from build123d import *

# Parameters (mm, degrees)
BASE_BLOCK_SKETCH_W       = 28
BASE_BLOCK_SKETCH_H       = 48
BASE_BLOCK_DEPTH          = 24
FORK_ARMS_DEPTH           = 10
FORK_ARC_CUT_SKETCH_R33_R = 16.5
FORK_ARC_CUT_DEPTH        = 20
EYE_START                 = -24
EYE_LUG_WITH_BORE_DEPTH   = 10


with BuildPart() as part:
    # Base Block Sketch → Base Block (new, symmetric)
    with BuildSketch(Plane.XY):
        with Locations((14, -24)):
            Rectangle(BASE_BLOCK_SKETCH_W, BASE_BLOCK_SKETCH_H)
    extrude(amount=BASE_BLOCK_DEPTH, both=True)

    # Fork Arms Sketch → Fork Arms (add, symmetric)
    with BuildSketch(Plane(origin=(0, -24, 0), x_dir=(1, 0, 0), z_dir=(0, 1, 0))):
        with BuildLine():
            Line((52, 24), (28, 24))
            Line((28, 24), (28, -24))
            Line((28, -24), (52, -24))
            ThreePointArc((52, -24), (76, 0), (52, 24))
        make_face()
    extrude(amount=FORK_ARMS_DEPTH, both=True)

    # Fork Arc Cut Sketch R33 → Fork Arc Cut (cut)
    with BuildSketch(Plane(origin=(0, -14, 0), x_dir=(1, 0, 0), z_dir=(0, 1, 0))):
        with Locations(Location((52, 0, 0), (0, 0, 270))):
            Circle(FORK_ARC_CUT_SKETCH_R33_R)
    extrude(amount=-FORK_ARC_CUT_DEPTH, mode=Mode.SUBTRACT)

    # Eye Lug Sketch → Eye Lug With Bore (add, symmetric)
    with BuildSketch(Plane.XY.offset(24).offset(EYE_START)):
        with BuildLine():
            Line((0, 0), (-32.031280577, 0))
            ThreePointArc((-32.031280577, 0), (-40.397880843, -1.279221568), (-48, -5))
            Line((-48, -5), (-20, -5))
            ThreePointArc((-20, -5), (-1, -24), (-20, -43))
            Line((-20, -43), (-48, -43))
            ThreePointArc((-48, -43), (-40.397880843, -46.720778432), (-32.031280577, -48))
            Line((-32.031280577, -48), (0, -48))
            Line((0, -48), (0, 0))
        make_face()
    extrude(amount=EYE_LUG_WITH_BORE_DEPTH, both=True)


solid = part.part
The listing builds one solid part. Answer for the finished solid, in the listing's coordinates (mm). A direction names the side the tool comes from. Give positions to 0.01 mm unless a question says otherwise; leave off trailing zeros. Write each loop counter-clockwise with the first axis right and the second up, starting at its lowest first coordinate (ties: lowest second). Pieces come first, ordered by that corner, then holes.
Item 1: Section C-C, the plane y = -24 is taken. Write down the section's boundary in (x, z), plus the area to 3 significant figures.
Item 2: Section B-B, the plane x = 45.5 is taken. Write down the section's boundary in (y, z), plus the area to 3 significant figures.
Item 3: Flat-ended cylindrical pins translate along their axes: P1, Ø1.5, axis at y = -18, z = 5.5, coming from the -X side; P2, Ø1, axis at y = -12, z = 16, coming from the +X side; P3, Ø15.5, axis at y = -16, z = -19.5, coming from the -X side; P4, Ø4, axis at x = -22, z = -13, coming from the -Y side. Find the tip coordinate at first contact, or state that the pin passes through.
Item 4: Section A-A, the plane z = -13 is taken. Write down the section's boundary in (x, y), plus the area to 3 significant figures.
Item 5: Which of the six approach directions +Z, -Z, +X, -X, +Y, -Y give full straight-line access (tool end or side, diameter ignored) to faces 5 (the flat face through (0, -24, 17)), 6 (the flat face through (36, -34, -6)), 7 (the flat face through (28, -7, 0))?
Item 6: Find the intervals of material crossed by line 1 along Z through (x, y) = (-1.5, -3.5); line 2 along X through (y, z) = (-26, 0); line 3 along Y through (x, z) = (69, -1), in increasing order.
Item 7: Section D-D, the plane x = 29.5 is taken. Write down the section's boundary in (y, z), plus the area to 3 significant figures.
Item 8: Determine the mould class of faces 1 (the flat face through (-34, -43, 0)), 2 (the flat face through (4, -48, 0)), 3 (the flat face through (36, -14, -6)), 4 (the flat face through (0, -24, -17)) for opening direction Y: released by +Y, released by -Y, zero draft, split by the parting line, or undercut.
Completed:
1. outline: (-1, -10) - (0, -10) - (0, -24) - (52, -24) arc R24 ccw to (52, 24) - (0, 24) - (0, 10) - (-1, 10) - close; hole circle Ø33 at (52, 0)
1. area: 2,570 mm2
2. outline: (-34, -24) - (-14, -24) - (-14, -15.17) - (-34, -15.17) - close; (-34, 15.17) - (-14, 15.17) - (-14, 24) - (-34, 24) - close
2. area: 353 mm2
3. P1: stops at x = -2.24
3. P2: stops at x = 28
3. P3: stops at x = 0
3. P4: passes through
4. outline: (0, -48) - (28, -48) - (28, -34) - (41.84, -34) - (41.84, -14) - (28, -14) - (28, 0) - (0, 0) - close; (62.16, -34) - (72.17, -34) - (72.17, -14) - (62.16, -14) - close
4. area: 1,820 mm2
5. face 5: +Z, -X, +Y, -Y
5. face 6: +Z, -Z, +X, -Y
5. face 7: +Z, -Z, +X, +Y
6. line 1: z = -10 to 10
6. line 2: x = -1.11 to 35.5, 68.5 to 76
6. line 3: y = -34 to -14
7. outline: (-34, -24) - (-14, -24) - (-14, 24) - (-34, 24) - close
7. area: 960 mm2
8. face 1: undercut
8. face 2: released by -Y
8. face 3: released by +Y
8. face 4: zero draft
